Source: three-view drawing plus pictorial views. Frame: mm from the lowest corner of the part. A direction names the side the tool comes from. Coordinates: 2 decimals unless noted, no trailing zeros. Write each loop counter-clockwise with the first axis right and the second up, starting at its lowest first coordinate (ties: lowest second). Pieces come first, ordered by that corner, then holes. Notation, with made-up numbers: (57.25, 37.5) -> (83.25, 37.5) arc R10 ccw to (83.25, 47.5) -> close; hole circle Ø7 at (-5, 37). An arc over 180 degrees is marked (long way). One line per item, written item: value.
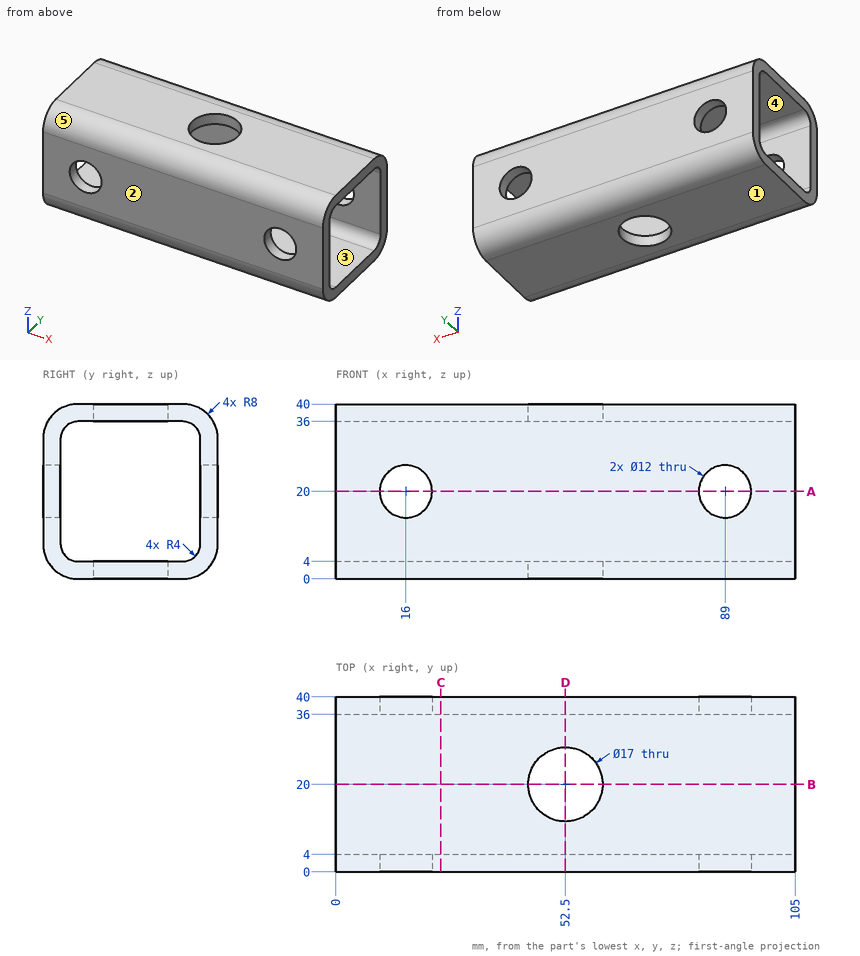
(1) First-contact query: pin 1 (4 mm diameter, centred on y = 33, z = 5, fed in from -X). Flat tip, straight axial feed; report the tip coordinate or a pass-through.
Responses:
pin 1: stops at x = 0
(2) Section C-C (x = 24). Return the cut outline in (y, z).
Responses:
outline: (0, 8) arc R8 ccw to (8, 0) -> (32, 0) arc R8 ccw to (40, 8) -> (40, 32) arc R8 ccw to (32, 40) -> (8, 40) arc R8 ccw to (0, 32) -> close; hole (4, 8) arc R4 ccw to (8, 4) -> (32, 4) arc R4 ccw to (36, 8) -> (36, 32) arc R4 ccw to (32, 36) -> (8, 36) arc R4 ccw to (4, 32) -> close
(3) Pull-direction query (Y, two-part tool) for the marked faces 1, 2 and 3; classes: released by +Y, released by -Y, zero draft, split by the parting line, or undercut.
Responses:
face 1: zero draft
face 2: released by -Y
face 3: undercut
(4) Line query: line 1 (X direction, y = 36.9, z = 20); line 2 (Y direction, x = 40.5, z = 25). Output: solid intervals per line, ascending. Write a range as [from, to].
Responses:
line 1: x = [0, 10], [22, 83], [95, 105]
line 2: y = [0, 4], [36, 40]
(5) Section B-B (y = 20). Return the cut outline in (x, z), then the cut area to 3 significant figures.
Responses:
outline: (0, 0) -> (44, 0) -> (44, 4) -> (0, 4) -> close; (0, 36) -> (44, 36) -> (44, 40) -> (0, 40) -> close; (61, 0) -> (105, 0) -> (105, 4) -> (61, 4) -> close; (61, 36) -> (105, 36) -> (105, 40) -> (61, 40) -> close
area: 704 mm2
(6) Reachability of the marked faces 4 and 5 from +Z, -Z, +X, -X, +Y, -Y: full face, straight path, thin tool, end or side. Return the list, or none.
Responses:
face 4: +X, -X
face 5: +Z, +X, -X, -Y
(7) Section A-A (z = 20). Return the cut outline in (x, y), then the cut area to 3 significant figures.
Responses:
outline: (0, 0) -> (10, 0) -> (10, 4) -> (0, 4) -> close; (0, 36) -> (10, 36) -> (10, 40) -> (0, 40) -> close; (22, 0) -> (83, 0) -> (83, 4) -> (22, 4) -> close; (22, 36) -> (83, 36) -> (83, 40) -> (22, 40) -> close; (95, 0) -> (105, 0) -> (105, 4) -> (95, 4) -> close; (95, 36) -> (105, 36) -> (105, 40) -> (95, 40) -> close
area: 648 mm2
(8) Section D-D (x = 52.5). Return the cut outline in (y, z).
Responses:
outline: (0, 8) arc R8 ccw to (8, 0) -> (11.5, 0) -> (11.5, 4) -> (8, 4) arc R4 cw to (4, 8) -> (4, 32) arc R4 cw to (8, 36) -> (11.5, 36) -> (11.5, 40) -> (8, 40) arc R8 ccw to (0, 32) -> close; (28.5, 0) -> (32, 0) arc R8 ccw to (40, 8) -> (40, 32) arc R8 ccw to (32, 40) -> (28.5, 40) -> (28.5, 36) -> (32, 36) arc R4 cw to (36, 32) -> (36, 8) arc R4 cw to (32, 4) -> (28.5, 4) -> close
